Design review of the part shown in the three views and the two pictorial views. Dimensions are in mm from the part's minimum x, y and z. Coordinates: 2 decimals unless noted, no trailing zeros. Loops run counter-clockwise (first coordinate to the right, second up) from the corner with the lowest first, then second, coordinate; pieces in that order, holes last.
Q1. Wall thickness on probe 1 along Y at (x, z) = (125, 5); probe 2 along Y at (x, z) = (122, 11.75); probe 3 along X at (y, z) = (149.5, 2.5): over which ranges is each line inside the solid? List them lowest first.
Q2. For P1, Ø4, axis at x = 69, z = 11.5, coming from the -Y side, flat-tipped, find the tip position at first contact; note if it passes through.
Q3. Add section A-A on y = 175. Give the boundary of the cut face in (x, z).
Q4. Add section C-C on z = 10. Give the boundary of the cut face in (x, y).
Q5. Add section B-B on x = 125. Give the boundary of the cut face in (y, z), and give its area (3 significant figures).
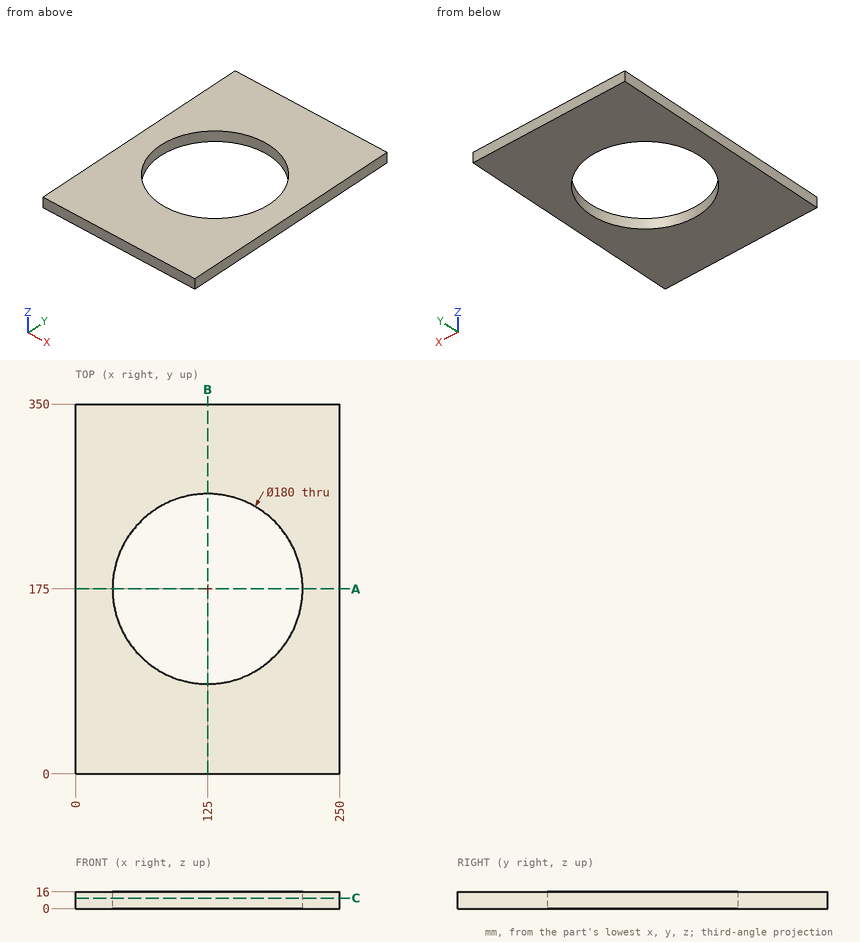
Entries:
1. probe 1: y = 0 to 85, 265 to 350
1. probe 2: y = 0 to 85.05, 264.95 to 350
1. probe 3: x = 0 to 38.69, 211.31 to 250
2. P1: stops at y = 0
3. outline: (0, 0) - (35, 0) - (35, 16) - (0, 16) - close; (215, 0) - (250, 0) - (250, 16) - (215, 16) - close
4. outline: (0, 0) - (250, 0) - (250, 350) - (0, 350) - close; hole circle Ø180 at (125, 175)
5. outline: (0, 0) - (85, 0) - (85, 16) - (0, 16) - close; (265, 0) - (350, 0) - (350, 16) - (265, 16) - close
5. area: 2,720 mm2
